Geometry check sheet. Reference: drawing and pictorial views, mm from the part's lowest x, y, z. A direction names the side the tool comes from. Round coordinates to 2 decimals unless told otherwise and drop trailing zeros. Write each loop counter-clockwise with the first axis right and the second up, starting at its lowest first coordinate (ties: lowest second). Pieces come first, ordered by that corner, then holes. Notation, with made-up numbers: (71, 64.25) -> (84, 64.25) arc R25 cw to (84, 100.25) -> close; hole circle Ø5 at (-21.75, 22). An arc over 180 degrees is marked (long way). Answer as a JSON object with one key per item and string values. Group by question number.
(1) Sectioned sample at C-C on z = 13.25. Record the cut outline in (x, y).
(2) Set-up check for the marked faces 1 and 2: record each of +Z, -Z, +X, -X, +Y, -Y from which the full face is reachable in a straight line by a thin tool's end or side.
(3) Gauge pin test, flat ends, axial feed: pin 1 Ø6 at (y, z) = (21, 17.5) entering from +X; pin 2 Ø5 at (y, z) = (39.5, 4.5) entering from -X; pin 3 Ø3 at (y, z) = (10.5, 16) entering from -X; pin 4 Ø13 at (x, y) = (23, 24) entering from -Z. Record the tip position at first contact, or that the pin passes through.
(4) Scan lines: L1, parallel to Y at x = 23, z = 4.5; L2, parallel to X at y = 23, z = 18.25 (1 decimal); L3, parallel to Z at x = 5.5, y = 13. Record each from-to range of solid material in increasing order. Write a range as from..to.
(5) Sectioned sample at A-A on x = 22.5. Record the cut outline in (y, z) (1 decimal), and give its area (3 significant figures).
(6) Draft check along Y on the marked faces 3, 4 and 5. Enter one of: released by +Y, released by -Y, zero draft, split by the parting line, or undercut.
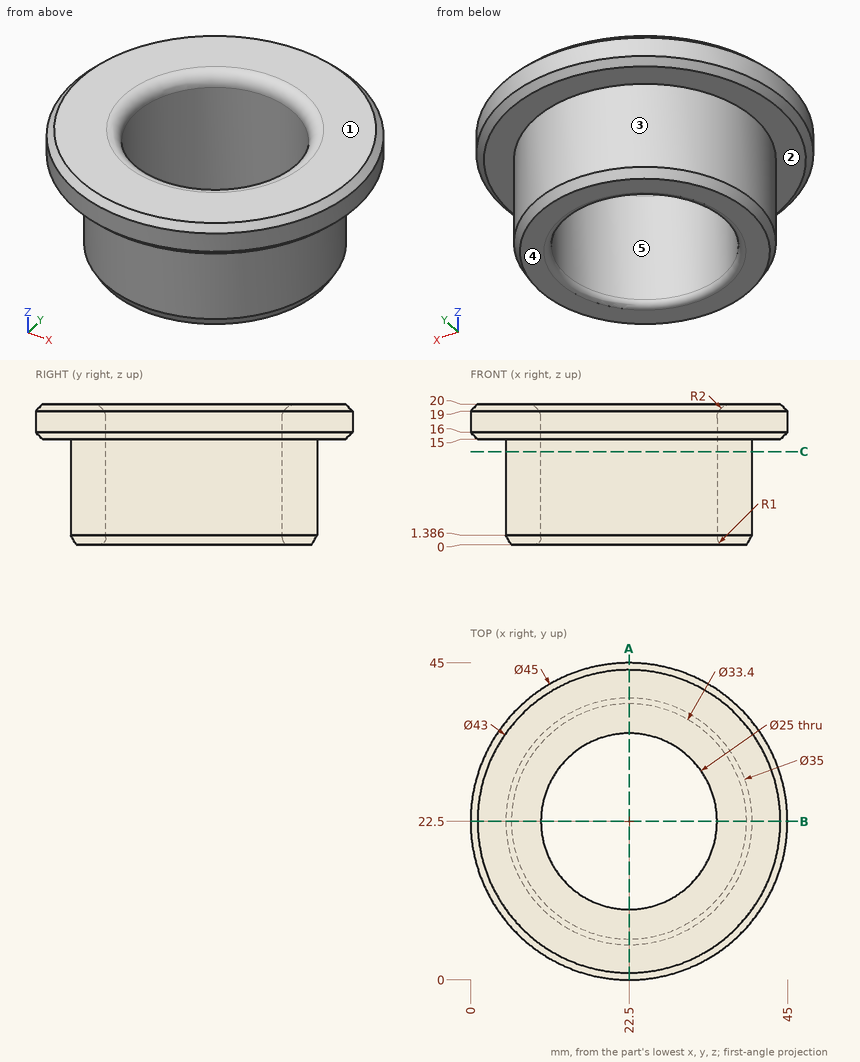
Computed values:
{
 "1": {"outline": "circle Ø35 at (22.5, 22.5); hole circle Ø25 at (22.5, 22.5)"},
 "2": {"face 1": "+Z, +X, -X, +Y, -Y", "face 2": "-Z"},
 "3": {"pin 1": "x = 45", "pin 2": "x = 12.7", "pin 3": "x = 2.6", "pin 4": "through"},
 "4": {"L1": "5.01..10.01, 34.99..39.99", "L2": "0..10, 35..45", "L3": "15..20"},
 "5": {"outline": "(0, 16) -> (1, 15) -> (5, 15) -> (5, 1.4) -> (5.8, 0) -> (9, 0) arc R1 ccw to (10, 1) -> (10, 18) arc R2 ccw to (8, 20) -> (1, 20) -> (0, 19) -> close; (35, 1) arc R1 ccw to (36, 0) -> (39.2, 0) -> (40, 1.4) -> (40, 15) -> (44, 15) -> (45, 16) -> (45, 19) -> (44, 20) -> (37, 20) arc R2 ccw to (35, 18) -> close", "area": "245 mm2"},
 "6": {"face 3": "split by the parting line", "face 4": "zero draft", "face 5": "undercut"}
}
